from build123d import *

# Parameters (mm, degrees)
SKETCH2_R           = 1.5
BOSS_EXTRUDE1_DEPTH = 1
BOSS_EXTRUDE2_DEPTH = 0.5
BOSS_EXTRUDE3_START = -0.1
SKETCH4_R           = 1.5
BOSS_EXTRUDE3_DEPTH = 0.1
BOSS_EXTRUDE5_START = -0.1
SKETCH5_R           = 1.5
BOSS_EXTRUDE5_DEPTH = 0.1


with BuildPart() as part:
    # Sketch2 → Boss-Extrude1 (new, symmetric)
    with BuildSketch(Plane.XY):
        with BuildLine():
            Line((-2.378864653, 11.189782176), (11.114395932, 37.671250283))
            ThreePointArc((11.114395932, 37.671250283), (16.00022062, 39.258705834), (17.587676171, 34.372881146))
            Line((17.587676171, 34.372881146), (4.094415586, 7.891413039))
            ThreePointArc((4.094415586, 7.891413039), (-0.791409102, 6.303957488), (-2.378864653, 11.189782176))
        make_face()
        with Locations((0.857775466, 9.540597607)):
            Circle(SKETCH2_R, mode=Mode.SUBTRACT)
        with Locations((14.351036052, 36.022065714)):
            Circle(SKETCH2_R, mode=Mode.SUBTRACT)
    extrude(amount=BOSS_EXTRUDE1_DEPTH, both=True)

    # Sketch3 → Boss-Extrude2 (add, symmetric)
    with BuildSketch(Plane.XY.offset(1)):
        with BuildLine():
            Line((1.637419261, 15.764424462), (9.676771623, 31.542216036))
            ThreePointArc((9.676771623, 31.542216036), (12.542887141, 32.47344695), (13.474118055, 29.607331431))
            Line((13.474118055, 29.607331431), (5.434765693, 13.829539858))
            ThreePointArc((5.434765693, 13.829539858), (2.568650175, 12.898308944), (1.637419261, 15.764424462))
        make_face()
    extrude(amount=BOSS_EXTRUDE2_DEPTH, both=True)

    # Sketch4 → Boss-Extrude3 (add)
    with BuildSketch(Plane.XY.offset(1).offset(BOSS_EXTRUDE3_START)):
        with Locations((0.857775466, 9.540597607)):
            Circle(SKETCH4_R)
    extrude(amount=BOSS_EXTRUDE3_DEPTH)

    # Sketch5 → Boss-Extrude5 (add)
    with BuildSketch(Plane.XY.offset(1).offset(BOSS_EXTRUDE5_START)):
        with Locations((14.351036052, 36.022065714)):
            Circle(SKETCH5_R)
    extrude(amount=BOSS_EXTRUDE5_DEPTH)


solid = part.part
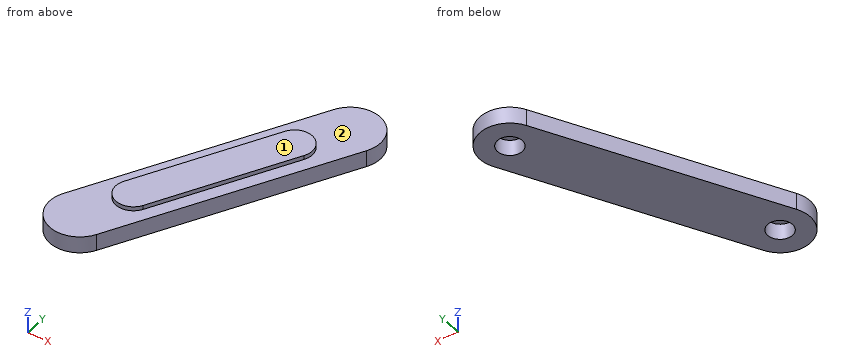
Source: CAD feature listing. Evaluate the final solid. Frame: model axes, mm. Face numbers are marked on the shaded views. A direction names the side the tool comes from. Coordinates: 2 decimals unless noted, no trailing zeros. Order: outer loops, then holes, each group sorted by start corner. A loop starts at its lowest first (then second) coordinate and runs counter-clockwise, first axis right, second up.
Item 1: Set-up query: the marked faces 1 and 2. Return all of +Z, -Z, +X, -X, +Y, -Y with unobstructed straight access to the full face (end or side cutting, diameter ignored); none if empty.
Output values:
face 1: +Z, +X, -X, +Y, -Y
face 2: +Z
Item 2: Cut plane D-D (x = 2). Return loops of the section in (y, z).
Output values:
outline: (6.09, -1) - (8.57, -1) - (8.57, 0.9) - (10.51, 0.9) - (10.51, -1) - (19.78, -1) - (19.78, 1) - (16.48, 1) - (16.48, 1.5) - (13.32, 1.5) - (13.32, 1) - (6.09, 1) - close
Item 3: First-contact query: P1, Ø2.5, axis at x = 0.86, y = 9.54, coming from the -Z side; P2, Ø5, axis at x = 14.35, y = 36.02, coming from the +Z side; P3, Ø1.5, axis at x = 6, z = -0.5, coming from the -Y side. Flat tips, straight axial feed; report the tip coordinate or a pass-through.
Output values:
P1: stops at z = 0.9
P2: stops at z = 1
P3: stops at y = 10.16
Item 4: Cut plane A-A (z = -0.45). Return loops of the section in (x, y).
Output values:
outline: (-2.38, 11.19) arc R3.63 ccw to (4.09, 7.89) - (17.59, 34.37) arc R3.63 ccw to (11.11, 37.67) - close; hole circle Ø3 at (0.86, 9.54); hole circle Ø3 at (14.35, 36.02)
Item 5: Material intervals for line 1 (Z direction, x = 14.25, y = 32.5); line 2 (Y direction, x = 1.75, z = -0.75); line 3 (X direction, y = 37, z = 0.6), sorted ascending.
Output values:
line 1: z = -1 to 1
line 2: y = 6.02 to 8.33, 10.75 to 19.29
line 3: x = 10.77 to 13.21, 15.49 to 17.85
Item 6: Cut plane C-C (y = 24). Return loops of the section in (x, z).
Output values:
outline: (4.15, -1) - (12.3, -1) - (12.3, 1) - (10.62, 1) - (10.62, 1.5) - (5.83, 1.5) - (5.83, 1) - (4.15, 1) - close
Item 7: Cut plane B-B (x = 9). Return loops of the section in (y, z).
Output values:
outline: (17.52, -1) - (33.52, -1) - (33.52, 1) - (30.21, 1) - (30.21, 1.5) - (20.83, 1.5) - (20.83, 1) - (17.52, 1) - close
